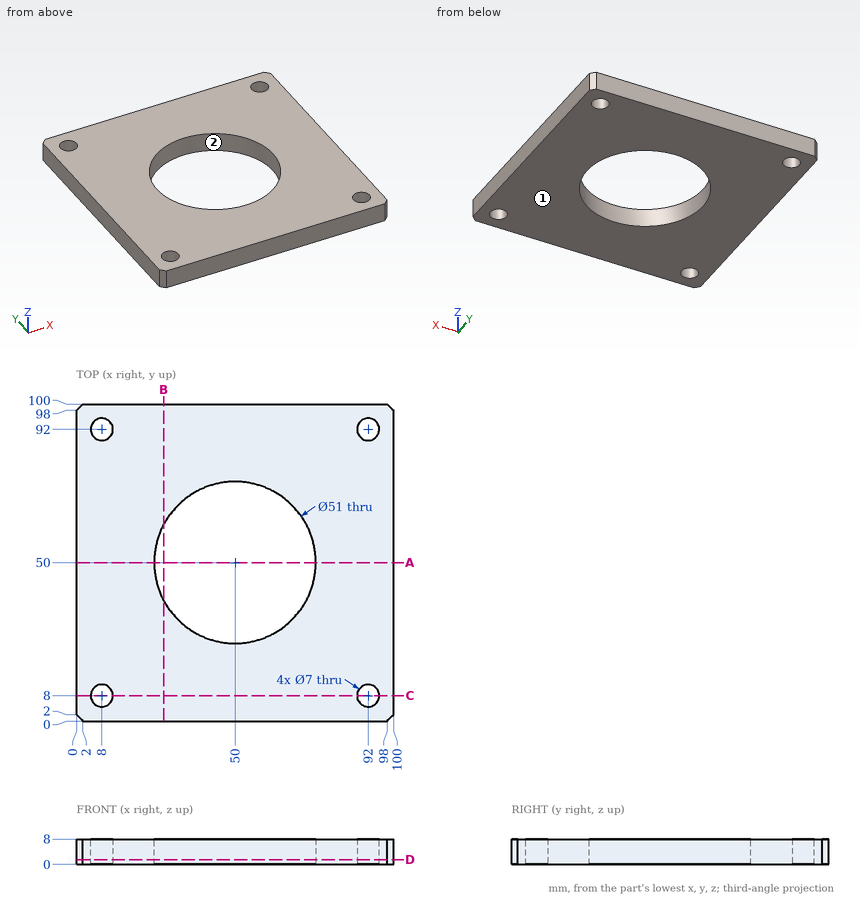
Can you work these out from the drawing? Everything is in mm from the part's minimum corner. Coordinates: 2 decimals unless noted, no trailing zeros. Loops run counter-clockwise (first coordinate to the right, second up) from the corner with the lowest first, then second, coordinate; pieces in that order, holes last.
1) Please list where these lines run through material, in increasing order: line 1 along Y through (x, z) = (93, 6.25); line 2 along X through (y, z) = (8, 3); line 3 along Y through (x, z) = (27.5, 5).
Reported:
line 1: y = 0 to 4.65, 11.35 to 88.65, 95.35 to 100
line 2: x = 0 to 4.5, 11.5 to 88.5, 95.5 to 100
line 3: y = 0 to 38, 62 to 100
2) Imagine slicing it at A-A (y = 50). List the corners of the cut face in (x, z) for me, and give its area (3 significant figures).
Reported:
outline: (0, 0) - (24.5, 0) - (24.5, 8) - (0, 8) - close; (75.5, 0) - (100, 0) - (100, 8) - (75.5, 8) - close
area: 392 mm2
3) Imagine slicing it at C-C (y = 8). List the corners of the cut face in (x, z) for me.
Reported:
outline: (0, 0) - (4.5, 0) - (4.5, 8) - (0, 8) - close; (11.5, 0) - (88.5, 0) - (88.5, 8) - (11.5, 8) - close; (95.5, 0) - (100, 0) - (100, 8) - (95.5, 8) - close
4) Will these pins go through, and if not, where does the flat tip stop? pin 1 Ø3 at (y, z) = (71.5, 2) entering from -X; pin 2 Ø4 at (x, y) = (8, 92) entering from -Z.
Reported:
pin 1: stops at x = 0
pin 2: passes through
5) Thinking about a two-plate mould opening in X: for the marked faces 1 and 2, which applies, released by +X, released by -X, zero draft, split by the parting line, or undercut?
Reported:
face 1: zero draft
face 2: undercut
6) Imagine slicing it at B-B (x = 27.5). List the corners of the cut face in (y, z) for me, and give its area (3 significant figures).
Reported:
outline: (0, 0) - (38, 0) - (38, 8) - (0, 8) - close; (62, 0) - (100, 0) - (100, 8) - (62, 8) - close
area: 608 mm2
7) Imagine slicing it at D-D (z = 1.5). List the corners of the cut face in (x, y) for me.
Reported:
outline: (0, 2) - (2, 0) - (98, 0) - (100, 2) - (100, 98) - (98, 100) - (2, 100) - (0, 98) - close; hole circle Ø7 at (8, 8); hole circle Ø7 at (8, 92); hole circle Ø51 at (50, 50); hole circle Ø7 at (92, 8); hole circle Ø7 at (92, 92)
